Geometry check sheet. Reference: the model listing, model coordinates, mm. A direction names the side the tool comes from. Round coordinates to 2 decimals unless told otherwise and drop trailing zeros. Loops run counter-clockwise (first coordinate to the right, second up) from the corner with the lowest first, then second, coordinate; pieces in that order, holes last. Notation, with made-up numbers: M -20,-39 L 27,-39 A19 cw 27,-18 Z; hole C 42,8.25 d7. An arc over 180 degrees is marked long. Use one line per item in the form item = value. Start each with the question number.
1. Cross-section at B-B (x = 87). Record the boundary of the cut face in (y, z).
2. Material ranges on line 1 (Z direction, x = 40.5, y = 19); line 2 (Y direction, x = 78.5, z = 2); line 3 (Z direction, x = 94, y = 49), recorded low to high.
3. Cross-section at C-C (z = 21.5). Record the boundary of the cut face in (x, y).
4. Set-up check for faces 1 (the flat face through (40, 25, 30)), 2 (the flat face through (79, 45, 25)), 3 (the flat face through (89, 51, 38)): record each of +Z, -Z, +X, -X, +Y, -Y from which the full face is reachable in a straight line by a thin tool's end or side.
5. Cross-section at D-D (y = 21). Record the boundary of the cut face in (x, z), then the cut area to 3 significant figures.
6. Draft check along X on faces 4 (the flat face through (97, 51, 36)), 5 (the flat face through (50, 35, 40)), 6 (the flat face through (107, 51, 41)), 7 (the flat face through (39, 25, 20)). Enter one of: pulls with the +X half, pulls with the -X half, needs draft (parallel to the pull), parting line crosses it, or undercut.
7. Cross-section at A-A (z = 14.5). Record the boundary of the cut face in (x, y).
8. Go/stop test with flat-tipped pins: pin 1 (11.5 mm diameter, centred on x = 31, y = 30.5, fed in from -Z); pin 2 (10 mm diameter, centred on y = 35, z = 10, fed in from -X); pin 3 (4 mm diameter, centred on y = 32.5, z = 29.5, fed in from +X). Record where each tip stops, or that it passes through.
```python
from build123d import *

# Parameters (mm, degrees)
BRACKET_BODY_50MM_DEPTH    = 50
STEP_POCKET_12MM_DEPTH     = 12
SLOT_CUT_12MM_DEPTH        = 12
TRIANGULAR_BOSS_30MM_DEPTH = 30
TRIANGULAR_CUT_20MM_DEPTH  = 20


with BuildPart() as part:
    # Bracket Body Profile → Bracket Body 50mm (new body)
    with BuildSketch(Plane.XY):
        Polygon((0, 0), (12, 0), (62, 0), (62, 45), (107, 45), (107, 57), (50, 57), (50, 12), (12, 12), (0, 12), align=None)
    extrude(amount=BRACKET_BODY_50MM_DEPTH)

    # Step Pocket Profile → Step Pocket 12mm (cut)
    with BuildSketch(Plane(origin=(0, 12, 0), x_dir=(1, 0, 0), z_dir=(0, 1, 0))):
        Polygon((0, -12), (0, 0), (12, 0), align=None)
        Polygon((0, -50), (0, -38), (12, -50), align=None)
    extrude(amount=-STEP_POCKET_12MM_DEPTH, mode=Mode.SUBTRACT)

    # Slot Cut Profile → Slot Cut 12mm (cut)
    with BuildSketch(Plane(origin=(0, 57, 0), x_dir=(1, 0, 0), z_dir=(0, 1, 0))):
        Polygon((107, -25), (107, -17), (97, -17), (97, -12), (82, -12), (82, -38), (97, -38), (97, -33), (107, -33), align=None)
    extrude(amount=-SLOT_CUT_12MM_DEPTH, mode=Mode.SUBTRACT)

    # Triangular Boss Profile → Triangular Boss 30mm (add)
    with BuildSketch(Plane.XY.offset(50)):
        Polygon((12, 12), (50, 12), (50, 57), align=None)
    extrude(amount=-TRIANGULAR_BOSS_30MM_DEPTH)

    # Triangular Cut Profile → Triangular Cut 20mm (cut)
    with BuildSketch(Plane.XY.offset(50)):
        Polygon((12, 12), (50, 57), (50, 12), align=None)
    extrude(amount=-TRIANGULAR_CUT_20MM_DEPTH, mode=Mode.SUBTRACT)


solid = part.part
```
Reported:
q1.outline = M 45,0 L 57,0 L 57,12 L 45,12 Z; M 45,38 L 57,38 L 57,50 L 45,50 Z
q2.line_1 = 20 to 30
q2.line_2 = 45 to 57
q2.line_3 = 0 to 12, 38 to 50
q3.outline = M 0,0 L 62,0 L 62,45 L 82,45 L 82,57 L 50,57 L 12,12 L 0,12 Z
q4.face_1 = +Z, -X, +Y
q4.face_2 = +Z, -Z, +X, -Y
q4.face_3 = +Y, -Y
q5.outline = M 19.6,20 L 50,20 L 50,0 L 62,0 L 62,50 L 50,50 L 50,30 L 19.6,30 Z
q5.area = 904 mm²
q6.face_4 = undercut
q6.face_5 = pulls with the -X half
q6.face_6 = pulls with the +X half
q6.face_7 = needs draft
q7.outline = M 0,0 L 62,0 L 62,45 L 82,45 L 82,57 L 50,57 L 50,12 L 0,12 Z; M 97,45 L 107,45 L 107,57 L 97,57 Z
q8.pin_1 = 20
q8.pin_2 = 50
q8.pin_3 = 62
